Geometry check sheet. Reference: the model listing, model coordinates, mm. A direction names the side the tool comes from. Round coordinates to 2 decimals unless told otherwise and drop trailing zeros. Order: outer loops, then holes, each group sorted by start corner. A loop starts at its lowest first (then second) coordinate and runs counter-clockwise, first axis right, second up. Notation, with made-up numbers: (57, 15.5) - (104, 15.5) arc R34 cw to (104, 45.5) - close; hole circle Ø3 at (54, 11.25). An arc over 180 degrees is marked (long way). Use a Markdown table: item, result. Add a question column.
(1) Gauge pin test, flat ends, axial feed: P1, Ø7, axis at y = 2.5, z = -3.5, coming from the -X side; P2, Ø10.5, axis at x = 79.65, z = 62.5, coming from the -Y side; P3, Ø11, axis at x = 13.5, y = -3, coming from the +Z side; P4, Ø5, axis at x = 101.5, y = 5.5, coming from the +Z side. Record the tip position at first contact, or that the pin passes through.
(2) Section check A-A on z = 18. Record the boundary of the cut face in (x, y).
(3) Mould release check, pull along X, two halves, no side actions. Record for faces 1 (the face through (104.445, -16.197, -46.062)), 2 (the face through (0, 9, 9)), 3 (the face through (20, -6, 1)): released by +X, released by -X, zero draft, split by the parting line, or undercut.
(4) Thickness scan on line 1 along X through (y, z) = (-11, -6); line 2 along X through (y, z) = (14.5, -13); line 3 along Y through (x, z) = (88, -47). Record the ranges inside material, lowest first. Write a range as [from, to].
(5) Section check B-B on y = -8.5. Record the boundary of the cut face in (x, z).
(6) Section check D-D on y = -15. Record the boundary of the cut face in (x, z), then the cut area to 3 significant figures.
(7) Access from +Z, -Z, +X, -X, +Y, -Y to the whole of each face (thin tool, end or side, straight path). Record for faces 4 (the face through (11, 0, 40)), 5 (the face through (3.49, 1.08, -4.88)), 6 (the face through (78.665, -16.303, 49.649)), 7 (the face through (11, 0, -40)).
(8) Section check C-C on x = 10.5. Record the boundary of the cut face in (y, z).
```python
from build123d import *

# Parameters (mm, degrees)
FRAME_BODY_DEPTH                  = 20
WINDOW_AND_HOLES_SKETCH_R         = 4
WINDOW_AND_HOLES_SKETCH_W         = 10
WINDOW_AND_HOLES_SKETCH_H         = 50
WINDOW_AND_FIXING_HOLES_CUT_DEPTH = 20
SIDE_SLOT_SKETCH_W                = 75
SIDE_SLOT_SKETCH_H                = 25
SIDE_SLOT_CUT_DEPTH               = 100
TOP_SLOT_SKETCH_W                 = 59
TOP_SLOT_SKETCH_H                 = 25
TOP_SLOT_CUT_DEPTH                = 20
COUNTERBORE_24_SKETCH_R           = 12
COUNTERBORE_24_DEPTH              = 3
HOLE_10_SKETCH_R                  = 5
HOLE_10_DEPTH                     = 30
CORNER_FILLETS_R9_R               = 9


with BuildPart() as part:
    # Frame Profile Sketch → Frame Body (new, symmetric)
    with BuildSketch(Plane(origin=(0, 0, 0), x_dir=(1, 0, 0), z_dir=(0, 1, 0))):
        with BuildLine():
            Line((25, 40), (74.996258615, 70.203420742))
            ThreePointArc((74.996258615, 70.203420742), (81.13209258, 71.377128003), (86.553849817, 68.273807903))
            Line((86.553849817, 68.273807903), (102.903849817, 48.723807903))
            ThreePointArc((102.903849817, 48.723807903), (104.459747288, 46.02126616), (105, 42.95))
            Line((105, 42.95), (105, -42.95))
            ThreePointArc((105, -42.95), (104.459747288, -46.02126616), (102.903849817, -48.723807903))
            Line((102.903849817, -48.723807903), (86.553849817, -68.273807903))
            ThreePointArc((86.553849817, -68.273807903), (81.13209258, -71.377128003), (74.996258615, -70.203420742))
            Line((74.996258615, -70.203420742), (25, -40))
            Line((25, -40), (0, -40))
            Line((0, -40), (0, 40))
            Line((0, 40), (25, 40))
        make_face()
    extrude(amount=FRAME_BODY_DEPTH, both=True)

    # Window and Holes Sketch → Window and Fixing Holes Cut (cut, symmetric)
    with BuildSketch(Plane(origin=(0, 0, 0), x_dir=(1, 0, 0), z_dir=(0, 1, 0))):
        with Locations(Location((79.65, 62.5, 0), (0, 0, 270))):
            Circle(WINDOW_AND_HOLES_SKETCH_R)
        with Locations(Location((96, 42.95, 0), (0, 0, 270))):
            Circle(WINDOW_AND_HOLES_SKETCH_R)
        with Locations(Location((96, -42.95, 0), (0, 0, 270))):
            Circle(WINDOW_AND_HOLES_SKETCH_R)
        with Locations(Location((79.65, -62.5, 0), (0, 0, 270))):
            Circle(WINDOW_AND_HOLES_SKETCH_R)
        Polygon((30.85, 31.850943236), (30.85, -31.850943236), (72.504579862, -57.015042236), (85, -42.074035282), (85, 42.074035282), (72.504579862, 57.015042236), align=None)
        with Locations((9, 0)):
            Rectangle(WINDOW_AND_HOLES_SKETCH_W, WINDOW_AND_HOLES_SKETCH_H)
    extrude(amount=WINDOW_AND_FIXING_HOLES_CUT_DEPTH, both=True, mode=Mode.SUBTRACT)

    # Side Slot Sketch → Side Slot Cut (cut, symmetric)
    with BuildSketch(Plane.XY):
        with Locations((57.5, 0)):
            Rectangle(SIDE_SLOT_SKETCH_W, SIDE_SLOT_SKETCH_H)
    extrude(amount=SIDE_SLOT_CUT_DEPTH, both=True, mode=Mode.SUBTRACT)

    # Top Slot Sketch → Top Slot Cut (cut)
    with BuildSketch(Plane(origin=(105, 0, 0), x_dir=(0, 0, -1), z_dir=(1, 0, 0))):
        with Locations((-42, 0)):
            Rectangle(TOP_SLOT_SKETCH_W, TOP_SLOT_SKETCH_H)
        with Locations((42, 0)):
            Rectangle(TOP_SLOT_SKETCH_W, TOP_SLOT_SKETCH_H)
    extrude(amount=-TOP_SLOT_CUT_DEPTH, mode=Mode.SUBTRACT)

    # Counterbore Ø24 Sketch → Counterbore Ø24 (cut)
    with BuildSketch(Plane.ZY):
        Circle(COUNTERBORE_24_SKETCH_R)
    extrude(amount=-COUNTERBORE_24_DEPTH, mode=Mode.SUBTRACT)

    # Hole Ø10 Sketch → Hole Ø10 (cut)
    with BuildSketch(Plane.ZY.offset(-3)):
        with Locations(Location((0, 0, 0), (0, 0, 270))):
            Circle(HOLE_10_SKETCH_R)
    extrude(amount=-HOLE_10_DEPTH, mode=Mode.SUBTRACT)

    # Corner Fillets R9
    corner_fillets_r9_edges = [part.edges().sort_by_distance(p)[0] for p in [
        (25, -16.25, -40),
        (25, -16.25, 40),
        (25, 16.25, -40),
        (25, 16.25, 40),
    ]]
    fillet(corner_fillets_r9_edges, radius=CORNER_FILLETS_R9_R)


solid = part.part
```
Check sheet entries:
| question | item | result |
|---|---|---|
| 1 | P1 | stops at x = 3 |
| 1 | P2 | stops at y = -20 |
| 1 | P3 | stops at z = 40 |
| 1 | P4 | stops at z = 12.5 |
| 2 | outline | (0, -20) - (4, -20) - (4, 20) - (0, 20) - close; (14, -20) - (30.85, -20) - (30.85, -12.5) - (20, -12.5) - (20, 12.5) - (30.85, 12.5) - (30.85, 20) - (14, 20) - close; (85, -20) - (105, -20) - (105, -12.5) - (85, -12.5) - close; (85, 12.5) - (105, 12.5) - (105, 20) - (85, 20) - close |
| 3 | face 1 | released by +X |
| 3 | face 2 | released by -X |
| 3 | face 3 | undercut |
| 4 | line 1 | x = [0, 4], [14, 20], [95, 105] |
| 4 | line 2 | x = [0, 4], [14, 30.85], [85, 105] |
| 4 | line 3 | y = [-20, -12.5], [12.5, 20] |
| 5 | outline | (0, -40) - (20, -40) - (20, 40) - (0, 40) - (0, 8.47) - (3, 8.47) - (3, -8.47) - (0, -8.47) - close; (95, -12.5) - (105, -12.5) - (105, 12.5) - (95, 12.5) - close; hole (4, -25) - (14, -25) - (14, 25) - (4, 25) - close |
| 6 | outline | (0, -40) - (22.49, -40) arc R9 cw to (27.15, -41.3) - (75, -70.2) arc R9 ccw to (86.55, -68.27) - (102.9, -48.72) arc R9 ccw to (105, -42.95) - (105, 42.95) arc R9 ccw to (102.9, 48.72) - (86.55, 68.27) arc R9 ccw to (75, 70.2) - (27.15, 41.3) arc R9 cw to (22.49, 40) - (0, 40) - close; hole (4, -25) - (14, -25) - (14, 25) - (4, 25) - close; hole (30.85, -31.85) - (72.5, -57.02) - (85, -42.07) - (85, 42.07) - (72.5, 57.02) - (30.85, 31.85) - close; hole circle Ø8 at (79.65, -62.5); hole circle Ø8 at (79.65, 62.5); hole circle Ø8 at (96, -42.95); hole circle Ø8 at (96, 42.95) |
| 6 | area | 5,610 mm2 |
| 7 | face 4 | +Z, -X, +Y, -Y |
| 7 | face 5 | -X |
| 7 | face 6 | +Y, -Y |
| 7 | face 7 | -Z, -X, +Y, -Y |
| 8 | outline | (-20, -40) - (20, -40) - (20, -25) - (-20, -25) - close; (-20, 25) - (20, 25) - (20, 40) - (-20, 40) - close |
